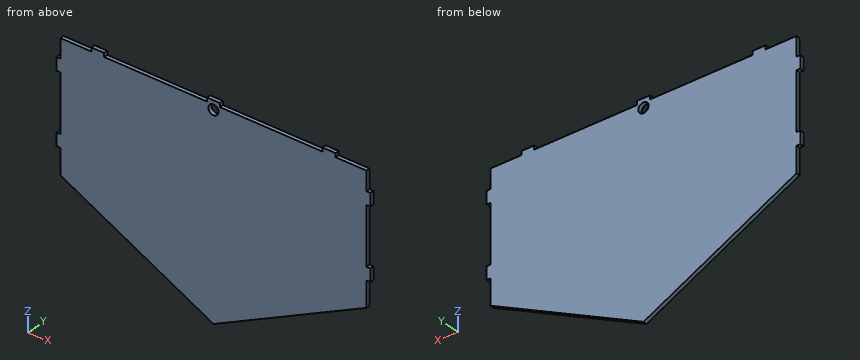
from build123d import *

# Parameters (mm, degrees)
BOSS_EXTRUDE1_DEPTH = 3
SKETCH3_W           = 3
SKETCH3_H           = 10
SKETCH3_W_2         = 10
SKETCH3_H_2         = 3
BOSS_EXTRUDE2_DEPTH = 3
SKETCH4_R           = 4
CUT_EXTRUDE1_DEPTH  = 165.295465549


with BuildPart() as part:
    # Sketch1 → Boss-Extrude1 (new body)
    with BuildSketch(Plane(origin=(0, 0, 0), x_dir=(1, 0, 0), z_dir=(0, 1, 0))):
        Polygon((-119, 50), (0, 110), (119, 50), (119, -50), (-119, -50), align=None)
    extrude(amount=BOSS_EXTRUDE1_DEPTH)

    # Sketch3 → Boss-Extrude2 (add)
    with BuildSketch(Plane(origin=(0, 3, 0), x_dir=(1, 0, 0), z_dir=(0, 1, 0))):
        with Locations((120.5, 25)):
            Rectangle(SKETCH3_W, SKETCH3_H)
        with Locations((120.5, -30)):
            Rectangle(SKETCH3_W, SKETCH3_H)
        with Locations((-120.5, -30)):
            Rectangle(SKETCH3_W, SKETCH3_H)
        with Locations((-120.5, 25)):
            Rectangle(SKETCH3_W, SKETCH3_H)
        with Locations((-90, -51.5)):
            Rectangle(SKETCH3_W_2, SKETCH3_H_2)
        with Locations((90, -51.5)):
            Rectangle(SKETCH3_W_2, SKETCH3_H_2)
        with Locations((0, -51.5)):
            Rectangle(SKETCH3_W_2, SKETCH3_H_2)
    extrude(amount=-BOSS_EXTRUDE2_DEPTH)

    # Sketch4 → Cut-Extrude1 (cut, through all)
    with BuildSketch(Plane(origin=(0, 3, 0), x_dir=(1, 0, 0), z_dir=(0, 1, 0))):
        with Locations(Location((0, -46, 0), (0, 0, 270))):
            Circle(SKETCH4_R)
    extrude(amount=-CUT_EXTRUDE1_DEPTH, mode=Mode.SUBTRACT)


solid = part.part
Could you check a few things on this model? Use its own coordinates, in mm. Round coordinates to 2 decimals unless told otherwise and drop trailing zeros. Order: outer loops, then holes, each group sorted by start corner. A loop starts at its lowest first (then second) coordinate and runs counter-clockwise, first axis right, second up.
Q1. Imagine slicing it at C-C, the plane x = 13. List the corners of the cut face in (y, z) for me.
Geometry says:
outline: (0, -103.45) - (3, -103.45) - (3, 50) - (0, 50) - close
Q2. I'm going to push flat-ended pins straight in: P1, Ø1.5, axis at x = -120, y = 1.5, coming from the -Z side; P2, Ø1.5, axis at y = 1.5, z = 52, coming from the -X side; P3, Ø0.9, axis at y = 1, z = 51, coming from the +X side. Where does each tip first touch, or does it pass through?
Geometry says:
P1: stops at z = -30
P2: stops at x = -95
P3: stops at x = 95
Q3. Imagine slicing it at A-A, the plane z = 46. List the corners of the cut face in (x, y) for me, then the cut area to 3 significant figures.
Geometry says:
outline: (-119, 0) - (-4, 0) - (-4, 3) - (-119, 3) - close; (4, 0) - (119, 0) - (119, 3) - (4, 3) - close
area: 690 mm2
Q4. Imagine slicing it at B-B, the plane z = -59. List the corners of the cut face in (x, y) for me, then the cut area to 3 significant figures.
Geometry says:
outline: (-101.15, 0) - (101.15, 0) - (101.15, 3) - (-101.15, 3) - close
area: 607 mm2
Q5. Please list where these lines run through material, in increasing order: probe 1 along X at (y, z) = (1.65, 46); probe 2 along X at (y, z) = (0.6, -8); probe 3 along Z at (x, y) = (63, 1.15).
Geometry says:
probe 1: x = -119 to -4, 4 to 119
probe 2: x = -119 to 119
probe 3: z = -78.24 to 50
